```python
from build123d import *

# Parameters (mm, degrees)
SKETCH1_R           = 8
BOSS_EXTRUDE1_DEPTH = 248
SKETCH2_R           = 4
BOSS_EXTRUDE2_DEPTH = 10
BOSS_EXTRUDE3_START = 6
SKETCH3_R           = 4
BOSS_EXTRUDE3_DEPTH = 6
CHAMFER1_SIZE       = 1


with BuildPart() as part:
    # Sketch1 → Boss-Extrude1 (new body)
    with BuildSketch(Plane.XY):
        Circle(SKETCH1_R)
    extrude(amount=BOSS_EXTRUDE1_DEPTH)

    # Sketch2 → Boss-Extrude2 (add)
    with BuildSketch(Plane(origin=(0, 0, 0), x_dir=(-1, 0, 0), z_dir=(0, 0, -1))):
        with Locations(Location((0, 0, 0), (0, 0, 180))):
            Circle(SKETCH2_R)
    extrude(amount=BOSS_EXTRUDE2_DEPTH)

    # Sketch3 → Boss-Extrude3 (add)
    with BuildSketch(Plane.XY.offset(248).offset(BOSS_EXTRUDE3_START)):
        Circle(SKETCH3_R)
    extrude(amount=-BOSS_EXTRUDE3_DEPTH)

    # Chamfer1
    chamfer1_edges = [part.edges().sort_by_distance(p)[0] for p in [
        (-4, 0, 254),
        (-4, 0, -10),
    ]]
    chamfer(chamfer1_edges, length=CHAMFER1_SIZE)


solid = part.part
```
Model file for the job. Use its own axes, mm. A direction names the side the tool comes from. Coordinates: 2 decimals unless noted, no trailing zeros. Write each loop counter-clockwise with the first axis right and the second up, starting at its lowest first coordinate (ties: lowest second). Pieces come first, ordered by that corner, then holes. Notation, with made-up numbers: (23, -8.5) - (81, -8.5) arc R29 cw to (81, 27.5) - close; hole circle Ø10 at (14.25, 39.25). An arc over 180 degrees is marked (long way). Use a Markdown table: item, result. Add a question column.
Item 1: Drop flat-ended pins along their axis: pin 1 (1.5 mm diameter, centred on x = 3, z = 29, fed in from +Y); pin 2 (1 mm diameter, centred on y = 2, z = 104, fed in from -X); pin 3 (2 mm diameter, centred on x = -5.5, y = 3.5, fed in from -Z). Give the stop position or say it passes through.
Item 2: Band-saw the part on C-C, the plane z = 66. Write the cut outline in (x, y), and give its area (3 significant figures).
Item 3: 3-axis set-ups, long thin cutter, end or side, ignore diameter. For faces 1 (the face through (-1.73, -7.81, 122.26)), 2 (the face through (-0.867, 3.905, -4.437)), 3 (the face through (-4, -2, 248)): which of +Z, -Z, +X, -X, +Y, -Y reach the whole face in a straight line?
Item 4: Band-saw the part on A-A, the plane x = 0. Write the cut outline in (y, z).
Item 5: Drill centre lines: line 1 along Z through (x, y) = (-5.25, -1.75); line 2 along Y through (x, z) = (5.5, 239); line 3 along Y through (x, z) = (4.25, 131). Where is each one in solid material? Low to high.
A:
| question | item | result |
|---|---|---|
| 1 | pin 1 | stops at y = 7.68 |
| 1 | pin 2 | stops at x = -7.86 |
| 1 | pin 3 | stops at z = 0 |
| 2 | outline | circle Ø16 at (0, 0) |
| 2 | area | 201 mm² |
| 3 | face 1 | +Z, -Z |
| 3 | face 2 | -Z |
| 3 | face 3 | +Z |
| 4 | outline | (-8, 0) - (-4, 0) - (-4, -9) - (-3, -10) - (3, -10) - (4, -9) - (4, 0) - (8, 0) - (8, 248) - (4, 248) - (4, 253) - (3, 254) - (-3, 254) - (-4, 253) - (-4, 248) - (-8, 248) - close |
| 5 | line 1 | z = 0 to 248 |
| 5 | line 2 | y = -5.81 to 5.81 |
| 5 | line 3 | y = -6.78 to 6.78 |
